Part model, mm, in its own coordinate system. Give positions to 0.01 mm unless a question says otherwise; leave off trailing zeros. Write each loop counter-clockwise with the first axis right and the second up, starting at its lowest first coordinate (ties: lowest second). Pieces come first, ordered by that corner, then holes. Notation, with made-up numbers: M 73.5,29.25 L 121.5,29.25 A15 ccw 121.5,53.25 Z; hole C -32,26.5 d11. An arc over 180 degrees is marked long. Use CSV: the item, a comma, the result in double quotes. Start each with the question number.
1. Band-saw the part on C-C, the plane x = 30. List the corners of the cut face in (y, z), then the cut area to 3 significant figures.
2. Band-saw the part on A-A, the plane y = 0. List the corners of the cut face in (x, z), then the cut area to 3 significant figures.
3. Drill centre lines: line 1 along Y through (x, z) = (90, 6.5); line 2 along X through (y, z) = (21, 6.75); line 3 along Y through (x, z) = (85, 5.75). Where is each one in solid material? Low to high. Write a range as from..to.
4. Band-saw the part on B-B, the plane x = -121.5. List the corners of the cut face in (y, z), then the cut area to 3 significant figures.
5. Drop flat-ended pins along their axis: pin 1 Ø5.5 at (x, y) = (30, 0) entering from +Z; pin 2 Ø10 at (x, y) = (90, 0) entering from +Z; pin 3 Ø2 at (x, y) = (-29.5, 38.5) entering from -Z. Give the stop position or say it passes through.
6. Band-saw the part on D-D, the plane x = 98.5. List the corners of the cut face in (y, z), then the cut area to 3 significant figures.
from build123d import *

# Parameters (mm, degrees)
SKETCH_1_W                = 260
SKETCH_1_H                = 80
EXTRUDE_1_DEPTH           = 10
CUT_EXTRUDE_1_REACH       = 138.382
SKETCH_2_R                = 20
CUT_EXTRUDE_2_REACH       = 138.382
SKETCH_3_R                = 12.5
HOLE_WIZARD_M5_1_D        = 4.2
HOLE_WIZARD_M5_1_DEPTH    = 12.4
HOLE_WIZARD_M5_1_TIP      = 1.2618073
HOLE_WIZARD_1_D           = 6.6
HOLE_WIZARD_1_CBORE_D     = 11
HOLE_WIZARD_1_CBORE_DEPTH = 6.8
HOLE_WIZARD_2_D           = 4.5
HOLE_WIZARD_2_DEPTH       = 10
HOLE_WIZARD_2_CBORE_D     = 8
HOLE_WIZARD_2_CBORE_DEPTH = 4.6
FILLET_1_R                = 5


with BuildPart() as part:
    # 草图1 → 凸台-拉伸1 (new body)
    with BuildSketch(Plane.XY):
        Rectangle(SKETCH_1_W, SKETCH_1_H)
    extrude(amount=EXTRUDE_1_DEPTH)

    # 草图2 → 切除-拉伸1 (cut, up to next)
    with BuildSketch(Plane.XY.offset(10), mode=Mode.PRIVATE) as cut_extrude_1_sk1:
        with Locations((-90, 0)):
            Circle(SKETCH_2_R)
    cut_extrude_1_tool1 = extrude(cut_extrude_1_sk1.sketch, amount=-CUT_EXTRUDE_1_REACH, mode=Mode.PRIVATE) & part.part
    # 草图2 → 切除-拉伸1 (cut, up to next)
    with BuildSketch(Plane.XY.offset(10), mode=Mode.PRIVATE) as cut_extrude_1_sk2:
        with Locations((-30, 0)):
            Circle(SKETCH_2_R)
    cut_extrude_1_tool2 = extrude(cut_extrude_1_sk2.sketch, amount=-CUT_EXTRUDE_1_REACH, mode=Mode.PRIVATE) & part.part
    add(cut_extrude_1_tool1.solids().sort_by_distance((-90, 0, 10))[0], mode=Mode.SUBTRACT)
    add(cut_extrude_1_tool2.solids().sort_by_distance((-30, 0, 10))[0], mode=Mode.SUBTRACT)

    # 草图3 → 切除-拉伸2 (cut, up to next)
    with BuildSketch(Plane.XY.offset(10), mode=Mode.PRIVATE) as cut_extrude_2_sk1:
        with Locations((30, -20)):
            Circle(SKETCH_3_R)
    cut_extrude_2_tool1 = extrude(cut_extrude_2_sk1.sketch, amount=-CUT_EXTRUDE_2_REACH, mode=Mode.PRIVATE) & part.part
    # 草图3 → 切除-拉伸2 (cut, up to next)
    with BuildSketch(Plane.XY.offset(10), mode=Mode.PRIVATE) as cut_extrude_2_sk2:
        with Locations((90, -20)):
            Circle(SKETCH_3_R)
    cut_extrude_2_tool2 = extrude(cut_extrude_2_sk2.sketch, amount=-CUT_EXTRUDE_2_REACH, mode=Mode.PRIVATE) & part.part
    # 草图3 → 切除-拉伸2 (cut, up to next)
    with BuildSketch(Plane.XY.offset(10), mode=Mode.PRIVATE) as cut_extrude_2_sk3:
        with Locations((30, 20)):
            Circle(SKETCH_3_R)
    cut_extrude_2_tool3 = extrude(cut_extrude_2_sk3.sketch, amount=-CUT_EXTRUDE_2_REACH, mode=Mode.PRIVATE) & part.part
    # 草图3 → 切除-拉伸2 (cut, up to next)
    with BuildSketch(Plane.XY.offset(10), mode=Mode.PRIVATE) as cut_extrude_2_sk4:
        with Locations((90, 20)):
            Circle(SKETCH_3_R)
    cut_extrude_2_tool4 = extrude(cut_extrude_2_sk4.sketch, amount=-CUT_EXTRUDE_2_REACH, mode=Mode.PRIVATE) & part.part
    add(cut_extrude_2_tool1.solids().sort_by_distance((30, -20, 10))[0], mode=Mode.SUBTRACT)
    add(cut_extrude_2_tool2.solids().sort_by_distance((90, -20, 10))[0], mode=Mode.SUBTRACT)
    add(cut_extrude_2_tool3.solids().sort_by_distance((30, 20, 10))[0], mode=Mode.SUBTRACT)
    add(cut_extrude_2_tool4.solids().sort_by_distance((90, 20, 10))[0], mode=Mode.SUBTRACT)

    # M5 螺纹孔1
    with Locations(Plane(origin=(130, 0, 0), x_dir=(0, 0, -1), z_dir=(1, 0, 0))):
        with Locations((-5, 30), (-5, -30)):
            Hole(HOLE_WIZARD_M5_1_D / 2, depth=HOLE_WIZARD_M5_1_DEPTH)
            with Locations((0, 0, -(HOLE_WIZARD_M5_1_DEPTH + HOLE_WIZARD_M5_1_TIP / 2))):  # 118° drill point
                Cone(0, HOLE_WIZARD_M5_1_D / 2, HOLE_WIZARD_M5_1_TIP, mode=Mode.SUBTRACT)

    # 打孔尺寸(%根据)内六角圆柱头螺钉的类型1 (through all)
    with Locations(Plane.XY.offset(10)):
        with Locations((90, 0), (30, 0)):
            CounterBoreHole(HOLE_WIZARD_1_D / 2, HOLE_WIZARD_1_CBORE_D / 2, HOLE_WIZARD_1_CBORE_DEPTH)

    # 打孔尺寸(%根据)内六角圆柱头螺钉的类型2
    with Locations(Plane(origin=(0, 0, 0), x_dir=(-1, 0, 0), z_dir=(0, 0, -1))):
        with Locations((30.500000316, -19.5), (30.500000316, 39.5), (121.500000316, 39.5), (121.500000316, -19.5)):
            CounterBoreHole(HOLE_WIZARD_2_D / 2, HOLE_WIZARD_2_CBORE_D / 2, HOLE_WIZARD_2_CBORE_DEPTH, depth=HOLE_WIZARD_2_DEPTH)

    # 圆角1
    fillet_1_edges = [part.edges().sort_by_distance(p)[0] for p in [
        (-130, 40, 5),
        (-130, -40, 5),
    ]]
    fillet(fillet_1_edges, radius=FILLET_1_R)


solid = part.part
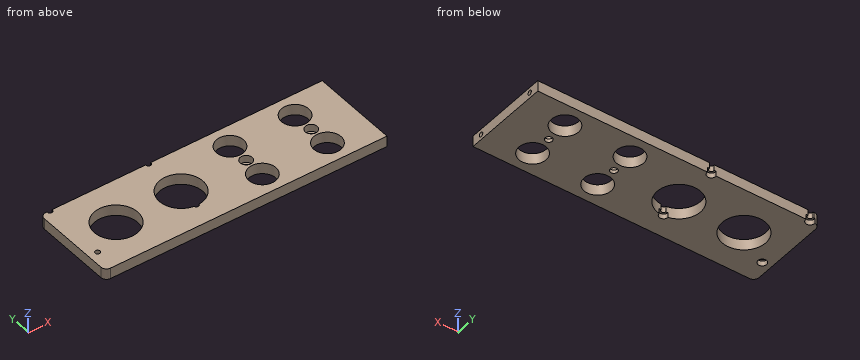
Output:
1,outline,"M -40,0 L -32.5,0 L -32.5,10 L -40,10 Z; M -7.5,0 L -3.3,0 L -3.3,3.2 L -5.5,3.2 L -5.5,10 L -7.5,10 Z; M 3.3,0 L 7.5,0 L 7.5,10 L 5.5,10 L 5.5,3.2 L 3.3,3.2 Z; M 32.5,0 L 40,0 L 40,10 L 32.5,10 Z"
1,area,"204 mm²"
2,outline,"M -130,0 L -110,0 L -110,10 L -130,10 Z; M -70,0 L -50,0 L -50,10 L -70,10 Z; M -10,0 L 26.7,0 L 26.7,3.2 L 24.5,3.2 L 24.5,10 L -10,10 Z; M 33.3,0 L 86.7,0 L 86.7,3.2 L 84.5,3.2 L 84.5,10 L 35.5,10 L 35.5,3.2 L 33.3,3.2 Z; M 93.3,0 L 130,0 L 130,10 L 95.5,10 L 95.5,3.2 L 93.3,3.2 Z"
2,area,"1,610 mm²"
3,line 1,"y = -40..-32.5, -7.5..-5.5, 5.5..7.5, 32.5..40"
3,line 2,"x = -130..17.54, 42.46..77.54, 102.46..130"
3,line 3,"y = -40..-31.46, -8.54..-2.29, 2.29..8.54, 31.46..40"
4,outline,"M -40,0 L -23.5,0 L -23.5,4.6 L -21.75,4.6 L -21.75,10 L -40,10 Z; M -17.25,4.6 L -15.5,4.6 L -15.5,0 L 35.5,0 L 35.5,4.6 L 37.25,4.6 L 37.25,10 L -17.25,10 Z"
4,area,"703 mm²"
5,pin 1,"passes through"
5,pin 2,"stops at z = 3.2"
5,pin 3,"stops at z = 4.6"
6,outline,"M -40,0 L -29.17,0 L -29.17,10 L -40,10 Z; M -10.83,0 L 10.83,0 L 10.83,10 L -10.83,10 Z; M 29.17,0 L 40,0 L 40,10 L 29.17,10 Z"
6,area,"433 mm²"
